Could you check a few things on this drawing? It's one solid part, dimensions in mm from its lowest x, y, z. Round coordinates to 2 decimals unless told otherwise and drop trailing zeros. Loops run counter-clockwise (first coordinate to the right, second up) from the corner with the lowest first, then second, coordinate; pieces in that order, holes last. Notation, with made-up numbers: (2, -40) -> (42, -40) arc R25 ccw to (42, -11) -> close; hole circle Ø10 at (-1.5, -25.75). An arc over 180 degrees is marked (long way). Write each question's results on one line, items separated by ' | '.
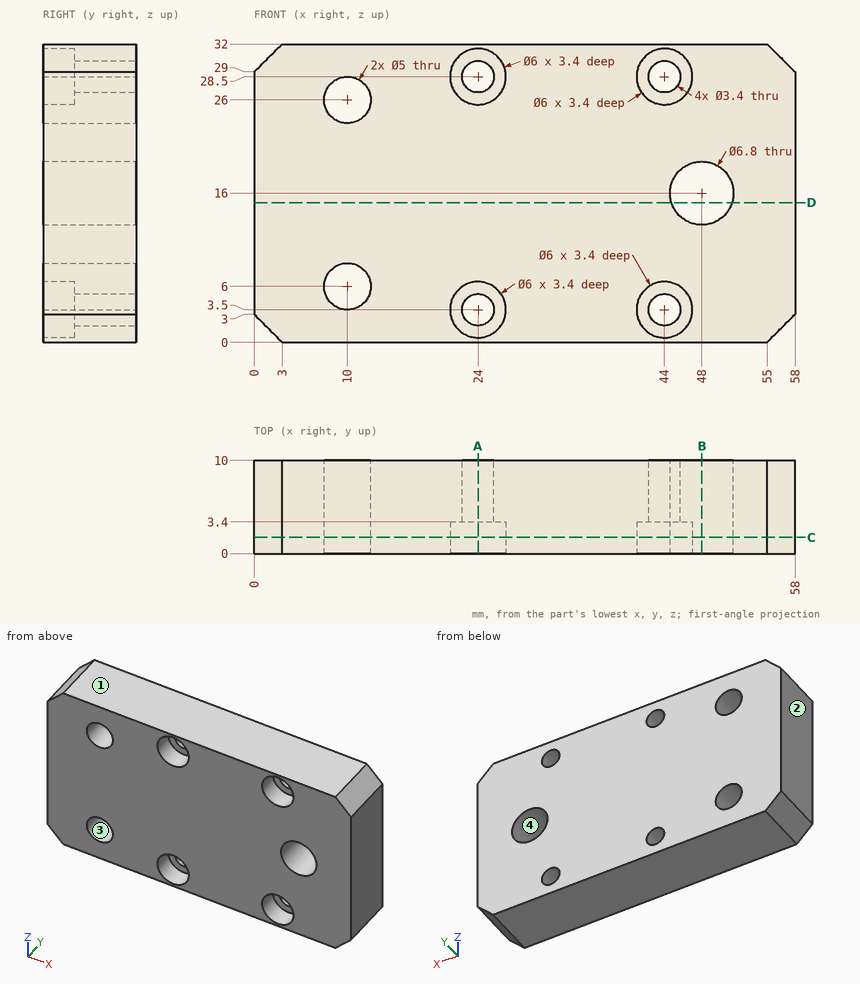
1) I want a section at C-C, the plane y = 1.75. Write out the boundary of the cut face in (x, z), plus the area to 3 significant figures.
Model answer:
outline: (0, 3) -> (3, 0) -> (55, 0) -> (58, 3) -> (58, 29) -> (55, 32) -> (3, 32) -> (0, 29) -> close; hole circle Ø5 at (10, 6); hole circle Ø5 at (10, 26); hole circle Ø6 at (24, 3.5); hole circle Ø6 at (24, 28.5); hole circle Ø6 at (44, 3.5); hole circle Ø6 at (44, 28.5); hole circle Ø6.8 at (48, 16) | area: 1,650 mm2
2) If we mould it in two halves opening along X, with no side actions, what happens to the marked faces 1, 2, 3 and 4? For each: released by +X, released by -X, zero draft, split by the parting line, or undercut.
Model answer:
face 1: zero draft | face 2: released by -X | face 3: undercut | face 4: undercut
3) I'm going to push flat-ended pins straight in: pin 1 (4 mm diameter, centred on x = 10, z = 6, fed in from -Y); pin 2 (4.5 mm diameter, centred on x = 24, z = 28.5, fed in from -Y). Where does each tip first touch, or does it pass through?
Model answer:
pin 1: passes through | pin 2: stops at y = 3.4
4) I need wall thicknesses on line 1 (Z direction, x = 24, y = 5.25); line 2 (Z direction, x = 44, y = 1.4); line 3 (X direction, y = 6.75, z = 2.5). Which ranges of each line are inside material? Lowest first, please.
Model answer:
line 1: z = 0 to 1.8, 5.2 to 26.8, 30.2 to 32 | line 2: z = 0 to 0.5, 6.5 to 25.5, 31.5 to 32 | line 3: x = 0.5 to 22.63, 25.37 to 42.63, 45.37 to 57.5
5) I want a section at A-A, the plane x = 24. Write out the boundary of the cut face in (y, z), plus the area to 3 significant figures.
Model answer:
outline: (0, 0) -> (10, 0) -> (10, 1.8) -> (3.4, 1.8) -> (3.4, 0.5) -> (0, 0.5) -> close; (0, 6.5) -> (3.4, 6.5) -> (3.4, 5.2) -> (10, 5.2) -> (10, 26.8) -> (3.4, 26.8) -> (3.4, 25.5) -> (0, 25.5) -> close; (0, 31.5) -> (3.4, 31.5) -> (3.4, 30.2) -> (10, 30.2) -> (10, 32) -> (0, 32) -> close | area: 234 mm2
6) I want a section at B-B, the plane x = 48. Write out the boundary of the cut face in (y, z), plus the area to 3 significant figures.
Model answer:
outline: (0, 0) -> (10, 0) -> (10, 12.6) -> (0, 12.6) -> close; (0, 19.4) -> (10, 19.4) -> (10, 32) -> (0, 32) -> close | area: 252 mm2
7) I want a section at D-D, the plane z = 15. Write out the boundary of the cut face in (x, y), plus the area to 3 significant figures.
Model answer:
outline: (0, 0) -> (44.75, 0) -> (44.75, 10) -> (0, 10) -> close; (51.25, 0) -> (58, 0) -> (58, 10) -> (51.25, 10) -> close | area: 515 mm2
